from build123d import *

# Parameters (mm, degrees)
BOX_PROFILE_SKETCH_R      = 1
BOX_SHELL_25MM_DEPTH      = 12.5
PARTITION_WALL_15MM_DEPTH = 7.5
SKETCH1_5_R               = 2.5
PARTITION_WALL_10MM_DEPTH = 5
NOTCH_CUT_4MM_DEPTH       = 65.468984791
NOTCH_CUT_4MM_DEPTH_BACK  = 4


with BuildPart() as part:
    # Box Profile Sketch → Box Shell 25mm (new, symmetric)
    with BuildSketch(Plane.XY):
        with BuildLine():
            Line((15, 30), (-15, 30))
            ThreePointArc((-15, 30), (-18.535533906, 28.535533906), (-20, 25))
            Line((-20, 25), (-20, -25))
            ThreePointArc((-20, -25), (-18.535533906, -28.535533906), (-15, -30))
            Line((-15, -30), (-7, -30))
            Line((-7, -30), (-3, -30))
            Line((-3, -30), (15, -30))
            ThreePointArc((15, -30), (18.535533906, -28.535533906), (20, -25))
            Line((20, -25), (20, 25))
            ThreePointArc((20, 25), (18.535533906, 28.535533906), (15, 30))
        make_face()
        with BuildLine():
            ThreePointArc((-18, 25), (-17.121320344, 27.121320344), (-15, 28))
            Line((-15, 28), (-3, 28))
            Line((-3, 28), (-3, 11.9990204))
            Line((-3, 11.9990204), (-3, 10.9990204))
            Line((-3, 10.9990204), (-3, -1.0009796))
            Line((-3, -1.0009796), (-3, -2.0009796))
            Line((-3, -2.0009796), (-3, -9))
            Line((-3, -9), (0, -9))
            Line((0, -9), (0, -28))
            Line((0, -28), (-3, -28))
            Line((-3, -28), (-7, -28))
            Line((-7, -28), (-15, -28))
            ThreePointArc((-15, -28), (-17.121320344, -27.121320344), (-18, -25))
            Line((-18, -25), (-18, -10.398895362))
            Line((-18, -10.398895362), (-18, -2.0009796))
            Line((-18, -2.0009796), (-18, -1.0009796))
            Line((-18, -1.0009796), (-18, 10.9990204))
            Line((-18, 10.9990204), (-18, 11.9990204))
            Line((-18, 11.9990204), (-18, 20.396936162))
            Line((-18, 20.396936162), (-18, 25))
        make_face(mode=Mode.SUBTRACT)
        with Locations((17.67963323, -26.519449845)):
            Circle(BOX_PROFILE_SKETCH_R, mode=Mode.SUBTRACT)
        with BuildLine():
            ThreePointArc((15, 28), (17.121320344, 27.121320344), (18, 25))
            Line((18, 25), (18, -23.676308898))
            ThreePointArc((18, -23.676308898), (15.270156966, -24.976559879), (15.23135699, -28))
            Line((15.23135699, -28), (2, -28))
            Line((2, -28), (2, -7))
            Line((2, -7), (-1, -7))
            Line((-1, -7), (-1, 28))
            Line((-1, 28), (15, 28))
        make_face(mode=Mode.SUBTRACT)
    extrude(amount=BOX_SHELL_25MM_DEPTH, both=True)

    # Sketch1_3 → Partition Wall 15mm (add, symmetric)
    with BuildSketch(Plane.XY):
        Polygon((-3, -2.0009796), (-3, -1.0009796), (-8.958312837, -1.0009796), (-18, -1.0009796), (-18, -2.0009796), (-8.925986332, -2.0009796), align=None)
        Polygon((-3, 10.9990204), (-3, 11.9990204), (-9.312399857, 11.9990204), (-18, 11.9990204), (-18, 10.9990204), (-9.312399857, 10.9990204), align=None)
    extrude(amount=PARTITION_WALL_15MM_DEPTH, both=True)

    # Sketch1_5 → Partition Wall 10mm (add, symmetric)
    # profile 1 of 3: a face of its own
    with BuildSketch(Plane.XY):
        with BuildLine():
            ThreePointArc((-9.312399857, 12.915792555), (-8.584814731, 22.545593209), (-18, 20.396936162))
            Line((-18, 20.396936162), (-18, 11.9990204))
            Line((-18, 11.9990204), (-9.312399857, 11.9990204))
            Line((-9.312399857, 11.9990204), (-9.312399857, 12.915792555))
        make_face()
        with Locations((-12.5, 17.9990204)):
            Circle(SKETCH1_5_R, mode=Mode.SUBTRACT)
    # profile 2 of 3: a face of its own
    with BuildSketch(Plane.XY):
        with BuildLine():
            Line((-9.312399857, 10.082248245), (-9.312399857, 10.9990204))
            Line((-9.312399857, 10.9990204), (-18, 10.9990204))
            Line((-18, 10.9990204), (-18, -1.0009796))
            Line((-18, -1.0009796), (-8.958312837, -1.0009796))
            Line((-8.958312837, -1.0009796), (-8.994851629, 0.129324835))
            ThreePointArc((-8.994851629, 0.129324835), (-6.503051462, 5.190353168), (-9.312399857, 10.082248245))
        make_face()
        with Locations((-12.5, 4.9990204)):
            Circle(SKETCH1_5_R, mode=Mode.SUBTRACT)
    # profile 3 of 3: a face of its own
    with BuildSketch(Plane.XY):
        with BuildLine():
            Line((-8.886875414, -3.210851133), (-8.925986332, -2.0009796))
            Line((-8.925986332, -2.0009796), (-18, -2.0009796))
            Line((-18, -2.0009796), (-18, -10.398895362))
            ThreePointArc((-18, -10.398895362), (-8.784213453, -12.71191691), (-8.886875414, -3.210851133))
        make_face()
        with Locations((-12.5, -8.0009796)):
            Circle(SKETCH1_5_R, mode=Mode.SUBTRACT)
    extrude(amount=PARTITION_WALL_10MM_DEPTH, both=True)

    # Notch Sketch → Notch Cut 4mm (cut, two sides: drawn at the far end of the back side and taken through both)
    with BuildSketch(Plane.XZ.offset(30).offset(-NOTCH_CUT_4MM_DEPTH_BACK)):
        with BuildLine():
            Line((-2, 7.5), (-2, 12.5))
            Line((-2, 12.5), (-10, 12.5))
            Line((-10, 12.5), (-10, 7.5))
            ThreePointArc((-10, 7.5), (-6, 3.5), (-2, 7.5))
        make_face()
    extrude(amount=NOTCH_CUT_4MM_DEPTH + NOTCH_CUT_4MM_DEPTH_BACK, mode=Mode.SUBTRACT)


solid = part.part
Source: CAD feature listing. Evaluate the final solid. Frame: model axes, mm. A direction names the side the tool comes from. Give positions to 0.01 mm unless a question says otherwise; leave off trailing zeros. Write each loop counter-clockwise with the first axis right and the second up, starting at its lowest first coordinate (ties: lowest second). Pieces come first, ordered by that corner, then holes. Notation, with made-up numbers: (80.25, 70.5) -> (138.25, 70.5) arc R10 cw to (138.25, 80.5) -> close; hole circle Ø8 at (-11, 88). An arc over 180 degrees is marked (long way). Write item = value, one per line.
Q1. Cut plane C-C on y = 23. Return loops of the section in (x, z).
Here are the results:
outline = (-20, -12.5) -> (-18, -12.5) -> (-18, 12.5) -> (-20, 12.5) -> close; (-15.82, -5) -> (-9.18, -5) -> (-9.18, 5) -> (-15.82, 5) -> close; (-3, -12.5) -> (-1, -12.5) -> (-1, 12.5) -> (-3, 12.5) -> close; (18, -12.5) -> (20, -12.5) -> (20, 12.5) -> (18, 12.5) -> close
Q2. First-contact query: pin 1 (0.8 mm diameter, centred on x = -9.5, y = -1.5, fed in from -Z); pin 2 (6 mm diameter, centred on x = -12.5, y = -10.5, fed in from +Z); pin 3 (3 mm diameter, centred on x = -8, y = 10, fed in from +Z). Flat tips, straight axial feed; report the tip coordinate or a pass-through.
Here are the results:
pin_1 = -7.5
pin_2 = 5
pin_3 = 7.5
Q3. Mould query, pull axis Y, two halves, no side actions, for faces 1 (the face through (16.68, -26.48, -0.18)), 2 (the face through (-12, -5, 5)), 3 (the face through (0, -30, 0)), 4 (the face through (-6.1, -29, 3.5)). Classes: +Y half, -Y half, draft (parallel to the pull), parting line (faces both ways), or undercut.
Here are the results:
face_1 = undercut
face_2 = undercut
face_3 = -Y half
face_4 = draft
Q4. Line query: line 1 (X direction, y = 1, z = 6.5); line 2 (Y direction, x = -12.5, z = 1.5); line 3 (X direction, y = -8, z = -10.5). Output: solid intervals per line, ascending. Write a range as from..to.
Here are the results:
line_1 = -20..-18, -3..-1, 18..20
line_2 = -30..-28, -14..-10.5, -5.5..2.5, 7.5..15.5, 20.5..24, 28..30
line_3 = -20..-18, -3..2, 18..20
Q5. Cut plane A-A on x = -17. Return loops of the section in (y, z).
Here are the results:
outline = (-29.58, -12.5) -> (-27.24, -12.5) -> (-27.24, 12.5) -> (-29.58, 12.5) -> close; (-11.97, -5) -> (-2, -5) -> (-2, -7.5) -> (-1, -7.5) -> (-1, -5) -> (11, -5) -> (11, -7.5) -> (12, -7.5) -> (12, -5) -> (21.97, -5) -> (21.97, 5) -> (12, 5) -> (12, 7.5) -> (11, 7.5) -> (11, 5) -> (-1, 5) -> (-1, 7.5) -> (-2, 7.5) -> (-2, 5) -> (-11.97, 5) -> close; (27.24, -12.5) -> (29.58, -12.5) -> (29.58, 12.5) -> (27.24, 12.5) -> close
Q6. Cut plane B-B on z = -8.25. Return loops of the section in (x, y), then the cut area to 3 significant figures.
Here are the results:
outline = (-20, -25) arc R5 ccw to (-15, -30) -> (15, -30) arc R5 ccw to (20, -25) -> (20, 25) arc R5 ccw to (15, 30) -> (-15, 30) arc R5 ccw to (-20, 25) -> close; hole (-18, -25) arc R3 ccw to (-15, -28) -> (0, -28) -> (0, -9) -> (-3, -9) -> (-3, 28) -> (-15, 28) arc R3 ccw to (-18, 25) -> close; hole (-1, -7) -> (2, -7) -> (2, -28) -> (15.23, -28) arc R2.86 cw to (18, -23.68) -> (18, 25) arc R3 ccw to (15, 28) -> (-1, 28) -> close; hole circle Ø2 at (17.68, -26.52)
area = 495 mm²
Q7. Reachability of faces 5 (the face through (-2, 0, 12.5)), 6 (the face through (-12, 15, 5)), 7 (the face through (-12, -5, -5)), 8 (the face through (9, -28, 0)), 9 (the face through (-2, -2, -12.5)) from +Z, -Z, +X, -X, +Y, -Y: full face, straight path, thin tool, end or side. Return the list, or none.
Here are the results:
face_5 = +Z, +X, -X, +Y, -Y
face_6 = +Z
face_7 = -Z
face_8 = +Z, -Z
face_9 = -Z, +X, -X, +Y, -Y
Q8. Cut plane D-D on x = -12.5. State how many separate pieces and enclosed holes the cut face has, then the cut area to 3 significant figures.
Here are the results:
separate_pieces = 6
enclosed_holes = 0
area = 340 mm²
